Work out the finished part from the listing and answer in its coordinate system (mm). A direction names the side the tool comes from. Round coordinates to 2 decimals unless told otherwise and drop trailing zeros. Write each loop counter-clockwise with the first axis right and the second up, starting at its lowest first coordinate (ties: lowest second). Pieces come first, ordered by that corner, then holes. Notation, with made-up numbers: M 64.5,86.25 L 83.5,86.25 A35 cw 83.5,124.25 Z; hole C -14,7.5 d2. An arc over 180 degrees is marked long. Answer in a Markdown table with one row per item.
```python
from build123d import *

# Parameters (mm, degrees)
BOSS_EXTRUDE1_DEPTH = 200


with BuildPart() as part:
    # Sketch1 → Boss-Extrude1 (new body)
    with BuildSketch(Plane.XY):
        Polygon((-17.319660113, 136.5), (17.319660113, 136.5), (22, 127.139320225), (22, 85.160679775), (17.319660113, 75.8), (-17.319660113, 75.8), (-22, 85.160679775), (-22, 127.139320225), align=None)
        Polygon((-14.229490169, 131.5), (14.229490169, 131.5), (17, 125.958980338), (17, 86.341019662), (14.229490169, 80.8), (-14.229490169, 80.8), (-17, 86.341019662), (-17, 125.958980338), align=None, mode=Mode.SUBTRACT)
    extrude(amount=BOSS_EXTRUDE1_DEPTH)


solid = part.part
```
1. Determine the mould class of faces 1 (the flat face through (-19.627, 80.415, 98.6)), 2 (the flat face through (-18, 109, 0)), 3 (the flat face through (-15.595, 83.532, 98.6)), 4 (the flat face through (19.693, 80.546, 98.6)) for opening direction X: released by +X, released by -X, zero draft, split by the parting line, or undercut.
Calculated:
| item | result |
|---|---|
| face 1 | released by -X |
| face 2 | zero draft |
| face 3 | undercut |
| face 4 | released by +X |
2. The part is cut by section A-A (x = 4). Determine the outline of the cut face in (y, z), plus the area to 3 significant figures.
Calculated:
| item | result |
|---|---|
| outline | M 75.8,0 L 80.8,0 L 80.8,200 L 75.8,200 Z; M 131.5,0 L 136.5,0 L 136.5,200 L 131.5,200 Z |
| area | 2,000 mm² |
3. The part is cut by section C-C (z = 177). Determine the outline of the cut face in (x, y), plus the area to 3 significant figures.
Calculated:
| item | result |
|---|---|
| outline | M -22,85.16 L -17.32,75.8 L 17.32,75.8 L 22,85.16 L 22,127.14 L 17.32,136.5 L -17.32,136.5 L -22,127.14 Z; hole M -17,86.34 L -14.23,80.8 L 14.23,80.8 L 17,86.34 L 17,125.96 L 14.23,131.5 L -14.23,131.5 L -17,125.96 Z |
| area | 890 mm² |
4. A tool of negligible diameter and unlimited length cuts with its end or side. For faces 5 (the flat face through (17, 106, 99)), 6 (the flat face through (0, 75.8, 99)), from which of +Z, -Z, +X, -X, +Y, -Y can it reach the whole face along a straight path? Write none if from no direction.
Calculated:
| item | result |
|---|---|
| face 5 | +Z, -Z |
| face 6 | +Z, -Z, +X, -X, -Y |
5. Consider line 1 along X through (y, z) = (101.5, 20); line 2 along Y through (x, z) = (-12, 68); line 3 along Y through (x, z) = (-16.5, 170.5). Determine where each line is inside the solid, lowest interval first. Write a range as from..to.
Calculated:
| item | result |
|---|---|
| line 1 | x = -22..-17, 17..22 |
| line 2 | y = 75.8..80.8, 131.5..136.5 |
| line 3 | y = 75.8..85.34, 126.96..136.5 |
6. Given pin 1 (10 mm diameter, centred on x = 5, y = 122.5, fed in from -Z), flat-ended and moving along its own axis, determine where the tip first touches the part or whether it passes through.
Calculated:
| item | result |
|---|---|
| pin 1 | passes through |
7. The part is cut by section B-B (y = 124). Determine the outline of the cut face in (x, z), plus the area to 3 significant figures.
Calculated:
| item | result |
|---|---|
| outline | M -22,0 L -17,0 L -17,200 L -22,200 Z; M 17,0 L 22,0 L 22,200 L 17,200 Z |
| area | 2,000 mm² |
